from build123d import *

# Parameters (mm, degrees)
EXTRUDE_1_DEPTH        = 50
EXTRUDE_1_2_DEPTH      = 3
CUT_EXTRUDE_1_REACH    = 640.784
SKETCH_3_R             = 4.1
HOLE_WIZARD_M8_1_D     = 6.8
HOLE_WIZARD_M8_1_DEPTH = 22.25
HOLE_WIZARD_M8_1_TIP   = 2.042926105
HOLE_WIZARD_M5_1_D     = 4.2


with BuildPart() as part:
    # 草图1 → Extrude 1 (new body)
    with BuildSketch(Plane.XY):
        Polygon((-500, 394), (-500, -150), (-300, -350), (500, -350), (500, 394), align=None)
        Polygon((-497, 391), (-497, -148.757359313), (-298.757359313, -347), (497, -347), (497, 391), align=None, mode=Mode.SUBTRACT)
    extrude(amount=EXTRUDE_1_DEPTH)

    # 草图2 → Extrude 1 2 (add)
    with BuildSketch(Plane.XY.offset(50)):
        Polygon((-500, -150), (-300, -350), (500, -350), (500, 394), (-500, 394), align=None)
    extrude(amount=EXTRUDE_1_2_DEPTH)

    # 草图3 → 切除-拉伸1 (cut, up to next)
    with BuildSketch(Plane.XY.offset(53), mode=Mode.PRIVATE) as cut_extrude_1_sk1:
        with Locations((386.5, 101.25)):
            Circle(SKETCH_3_R)
    cut_extrude_1_tool1 = extrude(cut_extrude_1_sk1.sketch, amount=-CUT_EXTRUDE_1_REACH, mode=Mode.PRIVATE) & part.part
    # 草图3 → 切除-拉伸1 (cut, up to next)
    with BuildSketch(Plane.XY.offset(53), mode=Mode.PRIVATE) as cut_extrude_1_sk2:
        with Locations((386.5, -15.25)):
            Circle(SKETCH_3_R)
    cut_extrude_1_tool2 = extrude(cut_extrude_1_sk2.sketch, amount=-CUT_EXTRUDE_1_REACH, mode=Mode.PRIVATE) & part.part
    add(cut_extrude_1_tool1.solids().sort_by_distance((386.5, 101.25, 53))[0], mode=Mode.SUBTRACT)
    add(cut_extrude_1_tool2.solids().sort_by_distance((386.5, -15.25, 53))[0], mode=Mode.SUBTRACT)

    # M8 螺纹孔1
    with Locations(Plane.ZY.offset(500)):
        with Locations((21, 284), (21, 254), (21, 54), (21, 24)):
            Hole(HOLE_WIZARD_M8_1_D / 2, depth=HOLE_WIZARD_M8_1_DEPTH)
            with Locations((0, 0, -(HOLE_WIZARD_M8_1_DEPTH + HOLE_WIZARD_M8_1_TIP / 2))):  # 118° drill point
                Cone(0, HOLE_WIZARD_M8_1_D / 2, HOLE_WIZARD_M8_1_TIP, mode=Mode.SUBTRACT)

    # M5 螺纹孔1 (through all)
    with Locations(Plane.XY.offset(53)):
        with Locations((447.014659804, -62), (480.514659804, -62), (447.014659804, 218), (480.514659804, 218)):
            Hole(HOLE_WIZARD_M5_1_D / 2)


solid = part.part
Geometry check sheet. Reference: the model listing, model coordinates, mm. A direction names the side the tool comes from. Coordinates: 2 decimals unless noted, no trailing zeros. Order: outer loops, then holes, each group sorted by start corner. A loop starts at its lowest first (then second) coordinate and runs counter-clockwise, first axis right, second up. Notation, with made-up numbers: (22.25, -22.5) - (29.25, -22.5) arc R36 cw to (29.25, 15.5) - close; hole circle Ø11 at (24, -8). An arc over 180 degrees is marked (long way). Answer in a Markdown table with one row per item. Add a question column.
1) Cross-section at C-C, the plane y = 341.5. Record the cut outline in (x, z).
2) Set-up check for faces 1 (the flat face through (94, -347, 25)), 2 (the flat face through (7, 394, 26)): record each of +Z, -Z, +X, -X, +Y, -Y from which the full face is reachable in a straight line by a thin tool's end or side.
3) Cross-section at B-B, the plane x = -127.5. Record the cut outline in (y, z), then the cut area to 3 significant figures.
4) Material ranges on line 1 along X through (y, z) = (218, 51); line 2 along Y through (x, z) = (386, 52); line 3 along X through (y, z) = (105, 39), recorded low to high. Write a range as [from, to].
5) Cross-section at A-A, the plane z = 33.5. Record the cut outline in (x, y).
6) Gauge pin test, flat ends, axial feed: P1, Ø6.5, axis at x = 386.5, y = 101.25, coming from the +Z side; P2, Ø6, axis at y = 24, z = 21, coming from the -X side; P3, Ø1, axis at x = 253.5, y = 182, coming from the -Z side; P4, Ø8, axis at y = -274.5, z = 6, coming from the -X side. Record the tip position at first contact, or that the pin passes through.
Check result:
| question | item | result |
|---|---|---|
| 1 | outline | (-500, 0) - (-497, 0) - (-497, 50) - (497, 50) - (497, 0) - (500, 0) - (500, 53) - (-500, 53) - close |
| 2 | face 1 | -Z |
| 2 | face 2 | +Z, -Z, +X, -X, +Y |
| 3 | outline | (-350, 0) - (-347, 0) - (-347, 50) - (391, 50) - (391, 0) - (394, 0) - (394, 53) - (-350, 53) - close |
| 3 | area | 2,530 mm² |
| 4 | line 1 | x = [-500, 444.91], [449.11, 478.41], [482.61, 500] |
| 4 | line 2 | y = [-350, -19.32], [-11.18, 97.18], [105.32, 394] |
| 4 | line 3 | x = [-500, -497], [497, 500] |
| 5 | outline | (-500, -150) - (-300, -350) - (500, -350) - (500, 394) - (-500, 394) - close; hole (-497, -148.76) - (-298.76, -347) - (497, -347) - (497, 391) - (-497, 391) - close |
| 6 | P1 | passes through |
| 6 | P2 | stops at x = 497 |
| 6 | P3 | stops at z = 50 |
| 6 | P4 | stops at x = -379.5 |
